Model file for the job. Use its own axes, mm. A direction names the side the tool comes from. Give positions to 0.01 mm unless a question says otherwise; leave off trailing zeros. Loops run counter-clockwise (first coordinate to the right, second up) from the corner with the lowest first, then second, coordinate; pieces in that order, holes last. Notation, with made-up numbers: M 23.25,81.5 L 63.25,81.5 A18 ccw 63.25,100.5 Z; hole C -33,45.5 d1. An arc over 180 degrees is marked long. Answer in a Markdown table with one row per item.
```python
from build123d import *

# Parameters (mm, degrees)
SKETCH1_R          = 12.05
SKETCH1_R_2        = 4.05
BOSS_EXTRU_1_DEPTH = 15
CHAMFER1_SIZE      = 1
CUT_EXTRUDE1_REACH = 24.703
SKETCH5_W          = 7
SKETCH5_H          = 40.880501257
SKETCH6_R          = 4
BOSS_EXTRU_4_DEPTH = 4


with BuildPart() as part:
    # Sketch1 → Boss.-Extru.1 (new body)
    with BuildSketch(Plane(origin=(0, 0, 0), x_dir=(1, 0, 0), z_dir=(0, 1, 0))):
        with Locations(Location((0, 0, 0), (0, 0, 270))):
            Circle(SKETCH1_R)
        with Locations(Location((0, 0, 0), (0, 0, 270))):
            Circle(SKETCH1_R_2, mode=Mode.SUBTRACT)
    extrude(amount=BOSS_EXTRU_1_DEPTH)

    # Chamfer1
    chamfer1_edges = [part.edges().sort_by_distance(p)[0] for p in [
        (0, 15, -12.05),
    ]]
    chamfer(chamfer1_edges, length=CHAMFER1_SIZE)

    # Sketch5 → Cut-Extrude1 (cut, up to next)
    with BuildSketch(Plane(origin=(0, 15, 0), x_dir=(1, 0, 0), z_dir=(0, 1, 0)), mode=Mode.PRIVATE) as cut_extrude1_sk1:
        with Locations((11.5, -1.662295536)):
            Rectangle(SKETCH5_W, SKETCH5_H)
    cut_extrude1_tool1 = extrude(cut_extrude1_sk1.sketch, amount=-CUT_EXTRUDE1_REACH, mode=Mode.PRIVATE) & part.part
    # Sketch5 → Cut-Extrude1 (cut, up to next)
    with BuildSketch(Plane(origin=(0, 15, 0), x_dir=(1, 0, 0), z_dir=(0, 1, 0)), mode=Mode.PRIVATE) as cut_extrude1_sk2:
        with Locations((-11.5, -1.662295536)):
            Rectangle(SKETCH5_W, SKETCH5_H)
    cut_extrude1_tool2 = extrude(cut_extrude1_sk2.sketch, amount=-CUT_EXTRUDE1_REACH, mode=Mode.PRIVATE) & part.part
    add(cut_extrude1_tool1.solids().sort_by_distance((11.5, 15, 1.662296))[0], mode=Mode.SUBTRACT)
    add(cut_extrude1_tool2.solids().sort_by_distance((-11.5, 15, 1.662296))[0], mode=Mode.SUBTRACT)

    # Sketch6 → Boss.-Extru.4 (add)
    with BuildSketch(Plane(origin=(8, 0, 0), x_dir=(0, 0, -1), z_dir=(1, 0, 0))):
        with BuildLine():
            Line((22.5, -2.5), (-22.5, -2.5))
            ThreePointArc((-22.5, -2.5), (-32.5, 7.5), (-22.5, 17.5))
            Line((-22.5, 17.5), (22.5, 17.5))
            ThreePointArc((22.5, 17.5), (32.5, 7.5), (22.5, -2.5))
        make_face()
        with Locations((23.579898115, 7.5)):
            Circle(SKETCH6_R, mode=Mode.SUBTRACT)
        with Locations(Location((-23.579898115, 7.5, 0), (0, 0, 180))):
            Circle(SKETCH6_R, mode=Mode.SUBTRACT)
    boss_extru_4 = extrude(amount=BOSS_EXTRU_4_DEPTH)

    # Mirror1: Boss.-Extru.4 across plane
    add(boss_extru_4.mirror(Plane(origin=(0, 0, 0), x_dir=(0, 0, 1), z_dir=(1, 0, 0))))


solid = part.part
```
Q1. 3-axis set-ups, long thin cutter, end or side, ignore diameter. For faces 1 (the face through (4, 0, 3)), 2 (the face through (-9.972, 5.968, -27.275)): which of +Z, -Z, +X, -X, +Y, -Y reach the whole face in a straight line?
Reported:
| item | result |
|---|---|
| face 1 | +Z, -Z, -Y |
| face 2 | +X, -X |
Q2. Probe probe 1 along X at (y, z) = (0.25, 23); probe 2 along X at (y, z) = (10.25, 0); probe 3 along Z at (x, y) = (-9.75, 6.5). List the from-to ranges inside material, lowest first.
Reported:
| item | result |
|---|---|
| probe 1 | -12 to -8, 8 to 12 |
| probe 2 | -12 to -4.05, 4.05 to 12 |
| probe 3 | -32.45 to -27.45, -19.71 to 19.71, 27.45 to 32.45 |
Q3. Saw through at B-B (y = 10.25). Give the number of separate pieces and of enclosed holes in the cut face, and give its area (3 significant figures).
Reported:
| item | result |
|---|---|
| separate pieces | 5 |
| enclosed holes | 1 |
| area | 724 mm² |
Q4. Saw through at A-A (x = 0). Give the cut face in (y, z).
Reported:
| item | result |
|---|---|
| outline | M 0,-12.05 L 14,-12.05 L 15,-11.05 L 15,-4.05 L 0,-4.05 Z; M 0,4.05 L 15,4.05 L 15,11.05 L 14,12.05 L 0,12.05 Z |
Q5. Mould opens along Y. For faces 3 (the face through (-12, 8, 0)), 4 (the face through (-9.972, 6.299, 27.395)), 5 (the face through (-10, 7.3, 32.5)) say: released by +Y, released by -Y, zero draft, split by the parting line, or undercut.
Reported:
| item | result |
|---|---|
| face 3 | zero draft |
| face 4 | undercut |
| face 5 | split by the parting line |
Q6. Drop flat-ended pins along their axis: pin 1 (3 mm diameter, centred on x = 7.5, y = 10, fed in from -Z); pin 2 (9 mm diameter, centred on y = 7.5, z = -23.58, fed in from -X); pin 3 (1.5 mm diameter, centred on x = 0, y = 8, fed in from +Z); pin 4 (5 mm diameter, centred on x = -2.5, z = 0, fed in from -Y). Give the stop position or say it passes through.
Reported:
| item | result |
|---|---|
| pin 1 | z = -32.44 |
| pin 2 | x = -12 |
| pin 3 | z = 12.05 |
| pin 4 | y = 0 |
Q7. Saw through at C-C (z = 0). Give the cut face in (x, y), and give its area (4 significant figures).
Reported:
| item | result |
|---|---|
| outline | M -12,-2.5 L -8,-2.5 L -8,0 L -4.05,0 L -4.05,15 L -8,15 L -8,17.5 L -12,17.5 Z; M 4.05,0 L 8,0 L 8,-2.5 L 12,-2.5 L 12,17.5 L 8,17.5 L 8,15 L 4.05,15 Z |
| area | 278.5 mm² |
Q8. Saw through at D-D (y = 1.5). Give the cut face in (x, z), and give its area (3 significant figures).
Reported:
| item | result |
|---|---|
| outline | M -12,-30.5 L -8,-30.5 L -8,-9.01 A12.05 ccw 8,-9.01 L 8,-30.5 L 12,-30.5 L 12,30.5 L 8,30.5 L 8,9.01 A12.05 ccw -8,9.01 L -8,30.5 L -12,30.5 Z; hole C 0,0 d8.1 |
| area | 791 mm² |
